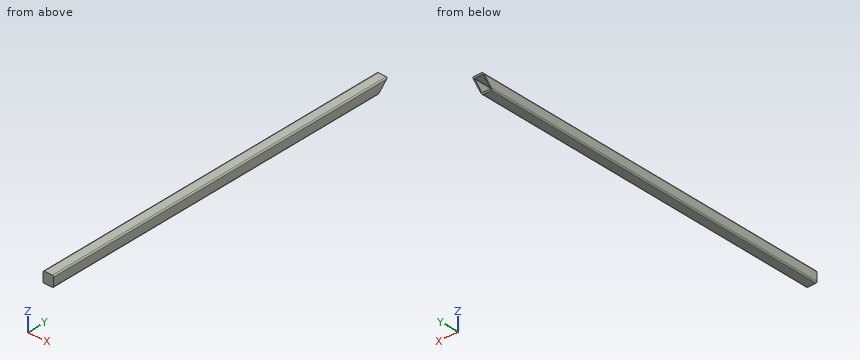
from build123d import *

# Parameters (mm, degrees)
EXTRUDE_1_DEPTH     = 1775
CUT_EXTRUDE_1_DEPTH = 1777.104710103
EXTRUDE_2_DEPTH     = 5
SKETCH_4_W          = 596.189257656
SKETCH_4_H          = 322.935847897
CUT_EXTRUDE_2_DEPTH = 1777.104710103
EXTRUDE_3_DEPTH     = 10


with BuildPart() as part:
    # 草图1 → 凸台-拉伸1 (new body)
    with BuildSketch(Plane(origin=(0, 0, 0), x_dir=(1, 0, 0), z_dir=(0, 1, 0))):
        with BuildLine():
            Line((-19, -12.278106509), (19, -12.278106509))
            ThreePointArc((19, -12.278106509), (23.242640687, -10.520747196), (25, -6.278106509))
            Line((25, -6.278106509), (25, 31.721893491))
            ThreePointArc((25, 31.721893491), (23.242640687, 35.964534178), (19, 37.721893491))
            Line((19, 37.721893491), (-19, 37.721893491))
            ThreePointArc((-19, 37.721893491), (-23.242640687, 35.964534178), (-25, 31.721893491))
            Line((-25, 31.721893491), (-25, -6.278106509))
            ThreePointArc((-25, -6.278106509), (-23.242640687, -10.520747196), (-19, -12.278106509))
        make_face()
        with BuildLine():
            Line((-19, -7.278106509), (19, -7.278106509))
            ThreePointArc((19, -7.278106509), (19.707106781, -6.98521329), (20, -6.278106509))
            Line((20, -6.278106509), (20, 31.721893491))
            ThreePointArc((20, 31.721893491), (19.707106781, 32.429000272), (19, 32.721893491))
            Line((19, 32.721893491), (-19, 32.721893491))
            ThreePointArc((-19, 32.721893491), (-19.707106781, 32.429000272), (-20, 31.721893491))
            Line((-20, 31.721893491), (-20, -6.278106509))
            ThreePointArc((-20, -6.278106509), (-19.707106781, -6.98521329), (-19, -7.278106509))
        make_face(mode=Mode.SUBTRACT)
    extrude(amount=EXTRUDE_1_DEPTH)

    # 草图2 → 切除-拉伸1 (cut, through all)
    with BuildSketch(Plane(origin=(25, 0, 0), x_dir=(0, 0, -1), z_dir=(1, 0, 0))):
        Polygon((-12.278106509, 1775), (37.721893491, 1775), (37.721893491, 1725), align=None)
    extrude(amount=-CUT_EXTRUDE_1_DEPTH, mode=Mode.SUBTRACT)

    # 草图3 → 凸台-拉伸2 (add)
    with BuildSketch(Plane.XZ):
        with BuildLine():
            Line((-25, 6.278106509), (-25, -31.721893491))
            ThreePointArc((-25, -31.721893491), (-23.242640687, -35.964534178), (-19, -37.721893491))
            Line((-19, -37.721893491), (19, -37.721893491))
            ThreePointArc((19, -37.721893491), (23.242640687, -35.964534178), (25, -31.721893491))
            Line((25, -31.721893491), (25, 6.278106509))
            ThreePointArc((25, 6.278106509), (23.242640687, 10.520747196), (19, 12.278106509))
            Line((19, 12.278106509), (-19, 12.278106509))
            ThreePointArc((-19, 12.278106509), (-23.242640687, 10.520747196), (-25, 6.278106509))
        make_face()
    extrude(amount=-EXTRUDE_2_DEPTH)

    # 草图4 → 切除-拉伸2 (cut, through all)
    with BuildSketch(Plane(origin=(25, 0, 0), x_dir=(0, 0, -1), z_dir=(1, 0, 0))):
        with Locations((-43.170849414, -111.467923949)):
            Rectangle(SKETCH_4_W, SKETCH_4_H)
    extrude(amount=-CUT_EXTRUDE_2_DEPTH, mode=Mode.SUBTRACT)

    # 草图5 → 凸台-拉伸3 (add)
    with BuildSketch(Plane.XZ.offset(-50)):
        with BuildLine():
            Line((-25, 6.278106509), (-25, -31.721893491))
            ThreePointArc((-25, -31.721893491), (-23.242640687, -35.964534178), (-19, -37.721893491))
            Line((-19, -37.721893491), (19, -37.721893491))
            ThreePointArc((19, -37.721893491), (23.242640687, -35.964534178), (25, -31.721893491))
            Line((25, -31.721893491), (25, 6.278106509))
            ThreePointArc((25, 6.278106509), (23.242640687, 10.520747196), (19, 12.278106509))
            Line((19, 12.278106509), (-19, 12.278106509))
            ThreePointArc((-19, 12.278106509), (-23.242640687, 10.520747196), (-25, 6.278106509))
        make_face()
    extrude(amount=-EXTRUDE_3_DEPTH)


solid = part.part
Design review of the part built by this model. Coordinates are the model's own, in mm. Give positions to 0.01 mm unless a question says otherwise; leave off trailing zeros. Write each loop counter-clockwise with the first axis right and the second up, starting at its lowest first coordinate (ties: lowest second). Pieces come first, ordered by that corner, then holes. Notation, with made-up numbers: M 39.25,58 L 86.25,58 A22 ccw 86.25,81 Z; hole C 44,66 d1. An arc over 180 degrees is marked long. Return JSON: item names as keys, results as strings. Group by question number.
Item 1: Take a section at C-C (z = -18.5). Give the boundary of the cut face in (x, y).
Item 2: Take a section at A-A (y = 1232.5). Give the boundary of the cut face in (x, z).
Item 3: Wall thickness on line 1 along Z through (x, y) = (-1.5, 1184.5); line 2 along X through (y, z) = (730.5, 3); line 3 along Z through (x, y) = (21, 1675): over which ranges is each line inside the solid? List them lowest first.
Item 4: Clearance check with a flat-ended pin moving along its axis: pin 1 Ø5 at (x, z) = (-5.5, -5.5) entering from +Y. State where the tip first meets the part, or that it passes through.
Item 5: Take a section at B-B (x = 1). Give the boundary of the cut face in (y, z).
Return value:
{
 "1": {"outline": "M -25,50 L 25,50 L 25,1744.22 L 20,1744.22 L 20,60 L -20,60 L -20,1744.22 L -25,1744.22 Z"},
 "2": {"outline": "M -25,-31.72 A6 ccw -19,-37.72 L 19,-37.72 A6 ccw 25,-31.72 L 25,6.28 A6 ccw 19,12.28 L -19,12.28 A6 ccw -25,6.28 Z; hole M -20,-31.72 A1 ccw -19,-32.72 L 19,-32.72 A1 ccw 20,-31.72 L 20,6.28 A1 ccw 19,7.28 L -19,7.28 A1 ccw -20,6.28 Z"},
 "3": {"line 1": "z = -37.72 to -32.72, 7.28 to 12.28", "line 2": "x = -25 to -20, 20 to 25", "line 3": "z = -37.38 to 11.93"},
 "4": {"pin 1": "stops at y = 60"},
 "5": {"outline": "M 50,-37.72 L 1725,-37.72 L 1730,-32.72 L 60,-32.72 L 60,7.28 L 1770,7.28 L 1775,12.28 L 50,12.28 Z"}
}
